from build123d import *

# Parameters (mm, degrees)
SKETCH1_R           = 4
BOSS_EXTRUDE1_DEPTH = 10
SKETCH2_R           = 9
BOSS_EXTRUDE2_DEPTH = 8
BOSS_EXTRUDE3_START = 12
SKETCH3_R           = 9
BOSS_EXTRUDE3_DEPTH = 12
BOSS_EXTRUDE4_START = 70
SKETCH4_R           = 4
BOSS_EXTRUDE4_DEPTH = 70
CHAMFER1_SIZE       = 0.5
SKETCH6_R           = 2.25
CUT_EXTRUDE2_DEPTH  = 10
CIRPATTERN1_COUNT   = 4
CHAMFER2_SIZE       = 0.5


with BuildPart() as part:
    # Sketch1 → Boss-Extrude1 (new body)
    with BuildSketch(Plane(origin=(0, 0, 0), x_dir=(1, 0, 0), z_dir=(0, 1, 0))):
        with Locations(Location((0, 0, 0), (0, 0, 270))):
            Circle(SKETCH1_R)
    extrude(amount=BOSS_EXTRUDE1_DEPTH)

    # Sketch2 → Boss-Extrude2 (add)
    with BuildSketch(Plane(origin=(0, 10, 0), x_dir=(1, 0, 0), z_dir=(0, 1, 0))):
        with Locations(Location((0, 0, 0), (0, 0, 270))):
            Circle(SKETCH2_R)
    extrude(amount=BOSS_EXTRUDE2_DEPTH)

    # Sketch3 → Boss-Extrude3 (add)
    with BuildSketch(Plane.XZ.offset(BOSS_EXTRUDE3_START)):
        with Locations(Location((0, 0, 0), (0, 0, 90))):
            Circle(SKETCH3_R)
    extrude(amount=-BOSS_EXTRUDE3_DEPTH)

    # Sketch4 → Boss-Extrude4 (add)
    with BuildSketch(Plane.XZ.offset(12).offset(BOSS_EXTRUDE4_START)):
        with Locations(Location((0, 0, 0), (0, 0, 270))):
            Circle(SKETCH4_R)
    extrude(amount=-BOSS_EXTRUDE4_DEPTH)

    # Chamfer1
    chamfer1_edges = [part.edges().sort_by_distance(p)[0] for p in [
        (0, -82, 4),
    ]]
    chamfer(chamfer1_edges, length=CHAMFER1_SIZE)

    # Sketch6 → Cut-Extrude2 (cut)
    with BuildSketch(Plane.XY):
        with Locations((0, -6)):
            Circle(SKETCH6_R)
    cut_extrude2 = extrude(amount=-CUT_EXTRUDE2_DEPTH, mode=Mode.SUBTRACT)

    # CirPattern1: Cut-Extrude2 ×4 about axis
    cirpattern1_axis = Axis((0, 18, 0), (0, -1, 0))
    for i in range(1, CIRPATTERN1_COUNT):
        add(cut_extrude2.rotate(cirpattern1_axis, i * 360 / CIRPATTERN1_COUNT), mode=Mode.SUBTRACT)

    # Chamfer2
    chamfer2_edges = [part.edges().sort_by_distance(p)[0] for p in [
        (0, 10, -9),
        (0, 18, -9),
        (0, 0, -9),
        (0, -12, -9),
    ]]
    chamfer(chamfer2_edges, length=CHAMFER2_SIZE)


solid = part.part
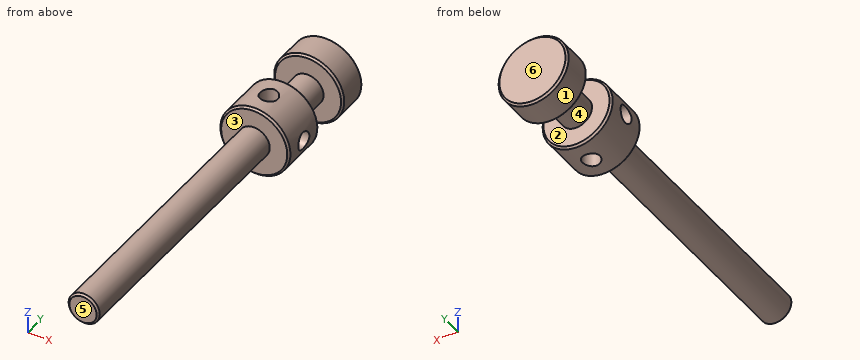
Can you work these out from the model? Positions are in its coordinate system, mm. Face numbers are marked on the shaded views. A direction names the side the tool comes from. Round coordinates to 2 decimals unless told otherwise and drop trailing zeros. Write each loop counter-clockwise with the first axis right and the second up, starting at its lowest first coordinate (ties: lowest second). Pieces come first, ordered by that corner, then holes. Notation, with made-up numbers: M 61.25,54.5 L 100.25,54.5 A23 ccw 100.25,64.5 Z; hole C 23.25,-24.75 d5. An arc over 180 degrees is marked long. Use CSV: the item, a comma, the result in double quotes.
(1) Imagine slicing it at B-B (z = 6). Count the separate pieces of the cut face and the enclosed holes in it, plus the area to 3 significant figures.
Check values:
separate pieces,"2"
enclosed holes,"1"
area,"251 mm^2"
(2) Imagine slicing it at A-A (y = -6). Write out the boundary of the cut face in (x, z), plus the area to 3 significant figures.
Check values:
outline,"M -8.71,-2.25 A9 ccw -2.25,-8.71 L -2.25,-2.25 Z; M -8.71,2.25 L -2.25,2.25 L -2.25,8.71 A9 ccw Z; M 2.25,-8.71 A9 ccw 8.71,-2.25 L 2.25,-2.25 Z; M 2.25,2.25 L 8.71,2.25 A9 ccw 2.25,8.71 Z"
area,"114 mm^2"
(3) We'd pull the mould along Y, two halves only. Please class the marked faces 4, 5 and 6: +Y half, -Y half, draft (parallel to the pull), parting line (faces both ways), or undercut.
Check values:
face 4,"undercut"
face 5,"-Y half"
face 6,"+Y half"
(4) I need wall thicknesses on line 1 along Y through (x, z) = (-6.5, 0); line 2 along Y through (x, z) = (0, -3.5); line 3 along Y through (x, z) = (4.5, 5.5). Which ranges of each line are inside material? Lowest first, please.
Check values:
line 1,"-12 to -8.25, -3.75 to 0, 10 to 18"
line 2,"-82 to -8.25, -3.75 to 18"
line 3,"-12 to 0, 10 to 18"
(5) On a 3-axis mill with a long thin cutter (end or side, diameter ignored), from which of +Z, -Z, +X, -X, +Y, -Y can I reach the whole of each face in a straight line? I mean the marked faces 1, 2 and 3. Say none if no direction works.
Check values:
face 1,"+Y, -Y"
face 2,"none"
face 3,"-Y"
(6) Imagine slicing it at C-C (y = -37). Write out the boundary of the cut face in (x, z).
Check values:
outline,"C 0,0 d8"
(7) I'm going to push flat-ended pins straight in: pin 1 (10 mm diameter, centred on y = -18, z = 0, fed in from -X); pin 2 (6 mm diameter, centred on x = 0, y = -6, fed in from +Z); pin 3 (6 mm diameter, centred on x = -3, y = -66.5, fed in from -Z); pin 4 (1.5 mm diameter, centred on y = -25, z = -3, fed in from +X). Where does each tip first touch, or does it pass through?
Check values:
pin 1,"x = -4"
pin 2,"z = 9"
pin 3,"z = -4"
pin 4,"x = 3.31"
